from build123d import *

# Parameters (mm, degrees)
SKETCH1_R           = 25
BOSS_EXTRUDE1_DEPTH = 50
SKETCH2_R           = 7.5
BOSS_EXTRUDE2_DEPTH = 25
CHAMFER1_SIZE       = 20
CHAMFER1_SIZE2      = 17
SKETCH3_R           = 6
CUT_EXTRUDE1_DEPTH  = 83.915619759
SKETCH4_R           = 21.453348456
CUT_EXTRUDE2_DEPTH  = 15


with BuildPart() as part:
    # Sketch1 → Boss-Extrude1 (new body)
    with BuildSketch(Plane(origin=(0, 0, 0), x_dir=(1, 0, 0), z_dir=(0, 1, 0))):
        with Locations(Location((0, 0, 0), (0, 0, 270))):
            Circle(SKETCH1_R)
    extrude(amount=BOSS_EXTRUDE1_DEPTH)

    # Sketch2 → Boss-Extrude2 (add)
    with BuildSketch(Plane(origin=(0, 50, 0), x_dir=(1, 0, 0), z_dir=(0, 1, 0))):
        with Locations(Location((0, 0, 0), (0, 0, 270))):
            Circle(SKETCH2_R)
    extrude(amount=BOSS_EXTRUDE2_DEPTH)

    # Chamfer1
    chamfer1_edges = [part.edges().sort_by_distance(p)[0] for p in [
        (0, 50, -25),
    ]]
    chamfer1_side = [part.faces().sort_by_distance(p)[0] for p in [
        (0, 25, -25),
    ]]
    chamfer(chamfer1_edges, length=CHAMFER1_SIZE, length2=CHAMFER1_SIZE2, reference=chamfer1_side[0])

    # Sketch3 → Cut-Extrude1 (cut, through all)
    with BuildSketch(Plane(origin=(0, 75, 0), x_dir=(1, 0, 0), z_dir=(0, 1, 0))):
        with Locations(Location((0, 0, 0), (0, 0, 270))):
            Circle(SKETCH3_R)
    extrude(amount=-CUT_EXTRUDE1_DEPTH, mode=Mode.SUBTRACT)

    # Sketch4 → Cut-Extrude2 (cut)
    with BuildSketch(Plane.XZ):
        with Locations(Location((0, 0, 0), (0, 0, 270))):
            Circle(SKETCH4_R)
    extrude(amount=-CUT_EXTRUDE2_DEPTH, mode=Mode.SUBTRACT)


solid = part.part
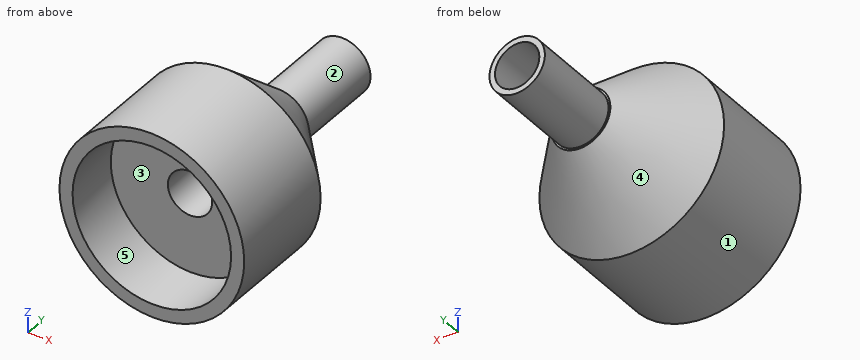
Build history of the part. All positions in model axes, mm. Face numbers are marked on the shaded views. A direction names the side the tool comes from. Coordinates: 2 decimals unless noted, no trailing zeros. Order: outer loops, then holes, each group sorted by start corner. A loop starts at its lowest first (then second) coordinate and runs counter-clockwise, first axis right, second up. Notation, with made-up numbers: (65.25, 20.5) - (107.25, 20.5) arc R25 cw to (107.25, 50.5) - close; hole circle Ø8 at (89, 18). An arc over 180 degrees is marked (long way). Write item = value, one per line. Start each with the question number.
1) Two-plate mould, pull along Z, no slides. Class the marked faces 4 and 5: pulls with the +Z half, pulls with the -Z half, needs draft (parallel to the pull), parting line crosses it, or undercut.
2) Saw through at A-A on z = 0. Write the cut outline in (x, y).
3) Wall check: line 1 along X through (y, z) = (58, 0); line 2 along X through (y, z) = (12, 0); line 3 along Z through (x, y) = (17, 10). Give the ranges that are in metal, low to high. Write a range as from..to.
4) 3-axis set-ups, long thin cutter, end or side, ignore diameter. For the marked faces 1, 2 and 3: which of +Z, -Z, +X, -X, +Y, -Y reach the whole face in a straight line?
5) Saw through at B-B on x = 0. Write the cut outline in (y, z).
6) Flat gauge pins, fed straight in: pin 1 Ø12 at (y, z) = (31, 8.5) entering from -X; pin 2 Ø13 at (x, z) = (-1.5, -1) entering from +Y; pin 3 Ø2 at (y, z) = (17.5, 5) entering from -X; pin 4 Ø10 at (x, z) = (-5, -10.5) entering from -Y. Where does each tip first touch, or does it go through?
From the geometry:
q1.face_4 = parting line crosses it
q1.face_5 = undercut
q2.outline = (-25, 0) - (-21.45, 0) - (-21.45, 15) - (-6, 15) - (-6, 75) - (-7.5, 75) - (-7.5, 50) - (-8, 50) - (-25, 30) - close; (6, 15) - (21.45, 15) - (21.45, 0) - (25, 0) - (25, 30) - (8, 50) - (7.5, 50) - (7.5, 75) - (6, 75) - close
q3.line_1 = -7.5..-6, 6..7.5
q3.line_2 = -25..-21.45, 21.45..25
q3.line_3 = -18.33..-13.09, 13.09..18.33
q4.face_1 = +Y, -Y
q4.face_2 = +Y
q4.face_3 = -Y
q5.outline = (0, -25) - (30, -25) - (50, -8) - (50, -7.5) - (75, -7.5) - (75, -6) - (15, -6) - (15, -21.45) - (0, -21.45) - close; (0, 21.45) - (15, 21.45) - (15, 6) - (75, 6) - (75, 7.5) - (50, 7.5) - (50, 8) - (30, 25) - (0, 25) - close
q6.pin_1 = -24.87
q6.pin_2 = 75
q6.pin_3 = -24.68
q6.pin_4 = 15
